from build123d import *

# Parameters (mm, degrees)
CLAMP_BASE_PROFILE_SKETCH_R = 7.5
CLAMP_BASE_PLATE_DEPTH      = 5
SLOTTED_UPRIGHT_TAB_DEPTH   = 10


with BuildPart() as part:
    # Clamp Base Profile Sketch → Clamp Base Plate (new, symmetric)
    with BuildSketch(Plane(origin=(0, 0, 0), x_dir=(1, 0, 0), z_dir=(0, 1, 0))):
        with BuildLine():
            Line((-25, -33.131068574), (-25, -11.749244617))
            Line((-25, -11.749244617), (25, -11.749244617))
            Line((25, -11.749244617), (25, -33.131068574))
            ThreePointArc((25, -33.131068574), (37.899800142, -58.991501114), (28.879478838, -86.446930784))
            ThreePointArc((28.879478838, -86.446930784), (21.733959657, -97.461955057), (17.711280988, -109.960245356))
            ThreePointArc((17.711280988, -109.960245356), (0.118395162, -124.74885524), (-17.667508621, -110.192954697))
            ThreePointArc((-17.667508621, -110.192954697), (-21.873782153, -97.444622756), (-29.130311117, -86.150576019))
            ThreePointArc((-29.130311117, -86.150576019), (-31.226426819, -83.403580628), (-33.064347445, -80.477536799))
            Line((-33.064347445, -80.477536799), (-20.312930357, -74.531453358))
            ThreePointArc((-20.312930357, -74.531453358), (21.751386889, -51.606406335), (-22.848639927, -69.093606636))
            Line((-22.848639927, -69.093606636), (-35.600057015, -75.039690077))
            ThreePointArc((-35.600057015, -75.039690077), (-36.839854324, -52.431244113), (-25, -33.131068574))
        make_face()
        with Locations(Location((0, -106.749244617, 0), (0, 0, 270))):
            Circle(CLAMP_BASE_PROFILE_SKETCH_R, mode=Mode.SUBTRACT)
    extrude(amount=CLAMP_BASE_PLATE_DEPTH, both=True)

    # Slotted Tab Profile Sketch → Slotted Upright Tab (add)
    with BuildSketch(Plane(origin=(0, 0, 11.749244617), x_dir=(-1, 0, 0), z_dir=(0, 0, -1))):
        with BuildLine():
            Line((-25, -5), (-25, 45))
            ThreePointArc((-25, 45), (0, 70), (25, 45))
            Line((25, 45), (25, -5))
            Line((25, -5), (-25, -5))
        make_face()
        with BuildLine():
            Line((7, 45), (7, 20))
            ThreePointArc((7, 20), (0, 13), (-7, 20))
            Line((-7, 20), (-7, 45))
            ThreePointArc((-7, 45), (0, 52), (7, 45))
        make_face(mode=Mode.SUBTRACT)
    extrude(amount=SLOTTED_UPRIGHT_TAB_DEPTH)


solid = part.part
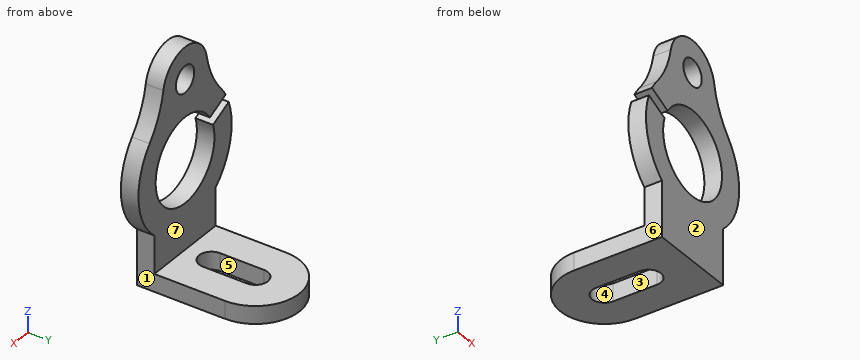
Check sheet for the modelled part. Datum: model origin and axes. Units: mm. Face numbers are marked on the shaded views. A direction names the side the tool comes from. Coordinates: 2 decimals unless noted, no trailing zeros. Loops run counter-clockwise (first coordinate to the right, second up) from the corner with the lowest first, then second, coordinate; pieces in that order, holes last. Notation, with made-up numbers: (-5, 48.5) -> (23, 48.5) arc R4 cw to (23, 52.5) -> close; hole circle Ø7 at (27, -8.5). An arc over 180 degrees is marked (long way). Write item = value, one per line. Start each with the question number.
1. Material ranges on line 1 (Z direction, x = -23.5, y = 46); line 2 (Y direction, x = -20, z = 99); line 3 (Y direction, x = 16, z = 10), recorded low to high.
2. Section check D-D on z = 49.5. Record the cut outline in (x, y).
3. Depth check by flat-ended pin: P1, Ø8, axis at y = 30, z = 7, coming from the -X side; P2, Ø23, axis at x = 15.5, z = 58.5, coming from the +Y side; P3, Ø25, axis at y = 11, z = 13, coming from the +X side. Enter the tip coordinate at first touch or a pass-through.
4. Tool access check on the marked faces 5, 6 and 7. Record the directions out of +Z, -Z, +X, -X, +Y, -Y that give a thin tool (end or side, any length) a straight path to the whole face; none if there is none.
5. Section check C-C on x = 0. Record the cut outline in (y, z).
6. Draft check along Y on the marked faces 1, 2, 3 and 4. Enter one of: released by +Y, released by -Y, zero draft, split by the parting line, or undercut.
7. Section check B-B on x = -11. Record the cut outline in (y, z), then the cut area to 3 significant figures.
8. Section check A-A on y = 37.5. Record the cut outline in (x, z), then the cut area to 3 significant figures.
Responses:
q1.line_1 = 1.75 to 11.75
q1.line_2 = -5 to 5
q1.line_3 = -5 to 64.21
q2.outline = (-35.97, -5) -> (-20.64, -5) -> (-20.64, 5) -> (-35.97, 5) -> close; (20.64, -5) -> (35.97, -5) -> (35.97, 5) -> (20.64, 5) -> close
q3.P1 = -25
q3.P2 = 5
q3.P3 = 25
q4.face_5 = +Z, -Z
q4.face_6 = -Z, -X, +Y, -Y
q4.face_7 = +Z, +X, -X, +Y
q5.outline = (-5, 1.75) -> (13, 1.75) -> (13, 11.75) -> (5, 11.75) -> (5, 37.75) -> (-5, 37.75) -> close; (-5, 85.75) -> (5, 85.75) -> (5, 99.25) -> (-5, 99.25) -> close; (-5, 114.25) -> (5, 114.25) -> (5, 124.75) -> (-5, 124.75) -> close; (52, 1.75) -> (70, 1.75) -> (70, 11.75) -> (52, 11.75) -> close
q6.face_1 = zero draft
q6.face_2 = released by -Y
q6.face_3 = undercut
q6.face_4 = undercut
q7.outline = (-5, 1.75) -> (67.45, 1.75) -> (67.45, 11.75) -> (5, 11.75) -> (5, 40.42) -> (-5, 40.42) -> close; (-5, 83.08) -> (5, 83.08) -> (5, 121) -> (-5, 121) -> close
q7.area = 1,390 mm2
q8.outline = (-25, 1.75) -> (-7, 1.75) -> (-7, 11.75) -> (-25, 11.75) -> close; (7, 1.75) -> (25, 1.75) -> (25, 11.75) -> (7, 11.75) -> close
q8.area = 360 mm2
